Geometry check sheet. Reference: the model listing, model coordinates, mm. A direction names the side the tool comes from. Coordinates: 2 decimals unless noted, no trailing zeros. Loops run counter-clockwise (first coordinate to the right, second up) from the corner with the lowest first, then second, coordinate; pieces in that order, holes last. Notation, with made-up numbers: (83, 28) - (104, 28) arc R15 cw to (104, 56) - close; hole circle Ø3 at (67, 65.25). An arc over 180 degrees is marked (long way). Write item = value, one per line. Start each with the question number.
from build123d import *

# Parameters (mm, degrees)
SKETCH1_W                    = 360
SKETCH1_H                    = 360
BOSS_EXTRUDE1_DEPTH          = 15
CHAMFER1_SIZE                = 10
F_9_0_9_DIAMETER_HOLE1_D     = 9
F_9_0_9_DIAMETER_HOLE1_DEPTH = 19.75
F_9_0_9_DIAMETER_HOLE1_TIP   = 2.703872786
SKETCH5_W                    = 90
SKETCH5_H                    = 100
CUT_EXTRUDE2_DEPTH           = 15
FILLET1_R                    = 5


with BuildPart() as part:
    # Sketch1 → Boss-Extrude1 (new body)
    with BuildSketch(Plane.XY):
        Rectangle(SKETCH1_W, SKETCH1_H)
    extrude(amount=BOSS_EXTRUDE1_DEPTH)

    # Chamfer1
    chamfer1_edges = [part.edges().sort_by_distance(p)[0] for p in [
        (-180, 180, 7.5),
        (180, 180, 7.5),
        (180, -180, 7.5),
        (-180, -180, 7.5),
    ]]
    chamfer(chamfer1_edges, length=CHAMFER1_SIZE)

    # Ø9.0 (9) Diameter Hole1
    with Locations(Plane.XY.offset(15)):
        with Locations((165, -45), (45, -45), (45, -165), (165, -165)):
            Hole(F_9_0_9_DIAMETER_HOLE1_D / 2, depth=F_9_0_9_DIAMETER_HOLE1_DEPTH)
            with Locations((0, 0, -(F_9_0_9_DIAMETER_HOLE1_DEPTH + F_9_0_9_DIAMETER_HOLE1_TIP / 2))):  # 118° drill point
                Cone(0, F_9_0_9_DIAMETER_HOLE1_D / 2, F_9_0_9_DIAMETER_HOLE1_TIP, mode=Mode.SUBTRACT)

    # Sketch5 → Cut-Extrude2 (cut)
    with BuildSketch(Plane.XY.offset(15)):
        with Locations((105, -105)):
            Rectangle(SKETCH5_W, SKETCH5_H)
    extrude(amount=-CUT_EXTRUDE2_DEPTH, mode=Mode.SUBTRACT)

    # Fillet1
    fillet1_edges = [part.edges().sort_by_distance(p)[0] for p in [
        (150, -55, 7.5),
        (150, -155, 7.5),
        (60, -155, 7.5),
        (60, -55, 7.5),
    ]]
    fillet(fillet1_edges, radius=FILLET1_R)


solid = part.part
(1) Sectioned sample at C-C on y = -112.5. Enter the section's corners in (x, z).
(2) Sectioned sample at A-A on x = 165. Enter the section's corners in (y, z).
(3) Draft check along Y on faces 1 (the face through (-2, 180, 7)), 2 (the face through (42.92, -48.99, 7.4)), 3 (the face through (-175, -175, 7)). Enter one of: pulls with the +Y half, pulls with the -Y half, needs draft (parallel to the pull), parting line crosses it, or undercut.
(4) Sectioned sample at D-D on z = 6. Enter the section's corners in (x, y), plus the area to 3 significant figures.
(5) Scan lines: line 1 (Y direction, x = 45, z = 11.75); line 2 (Y direction, x = 101, z = 13); line 3 (X direction, y = -71, z = 7.5). Record each from-to range of solid material in increasing order.
(6) Sectioned sample at B-B on y = -165. Enter the section's corners in (x, z).
(7) Tool access check on faces 4 (the face through (180, -2, 7)), 5 (the face through (60, -106, 8)). Record the directions out of +Z, -Z, +X, -X, +Y, -Y that give a thin tool (end or side, any length) a straight path to the whole face; none if there is none.
Working result:
q1.outline = (-180, 0) - (60, 0) - (60, 15) - (-180, 15) - close; (150, 0) - (180, 0) - (180, 15) - (150, 15) - close
q2.outline = (-180, 0) - (-169.5, 0) - (-169.5, 15) - (-180, 15) - close; (-160.5, 0) - (-49.5, 0) - (-49.5, 15) - (-160.5, 15) - close; (-40.5, 0) - (180, 0) - (180, 15) - (-40.5, 15) - close
q3.face_1 = pulls with the +Y half
q3.face_2 = undercut
q3.face_3 = pulls with the -Y half
q4.outline = (-180, -170) - (-170, -180) - (170, -180) - (180, -170) - (180, 170) - (170, 180) - (-170, 180) - (-180, 170) - close; hole circle Ø9 at (45, -165); hole circle Ø9 at (45, -45); hole (60, -150) arc R5 ccw to (65, -155) - (145, -155) arc R5 ccw to (150, -150) - (150, -60) arc R5 ccw to (145, -55) - (65, -55) arc R5 ccw to (60, -60) - close; hole circle Ø9 at (165, -165); hole circle Ø9 at (165, -45)
q4.area = 120,000 mm2
q5.line_1 = -180 to -169.5, -160.5 to -49.5, -40.5 to 180
q5.line_2 = -180 to -155, -55 to 180
q5.line_3 = -180 to 60, 150 to 180
q6.outline = (-180, 0) - (40.5, 0) - (40.5, 15) - (-180, 15) - close; (49.5, 0) - (160.5, 0) - (160.5, 15) - (49.5, 15) - close; (169.5, 0) - (180, 0) - (180, 15) - (169.5, 15) - close
q7.face_4 = +Z, -Z, +X, +Y, -Y
q7.face_5 = +Z, -Z
